```python
from build123d import *

# Parameters (mm, degrees)
SKETCH_1_W          = 5
SKETCH_1_H          = 300
EXTRUDE_1_DEPTH     = 60
SKETCH_2_R          = 5
CUT_EXTRUDE_1_DEPTH = 20


with BuildPart() as part:
    # 草图1 → 凸台-拉伸1 (new body)
    with BuildSketch(Plane.XY):
        Rectangle(SKETCH_1_W, SKETCH_1_H)
    extrude(amount=EXTRUDE_1_DEPTH)

    # 草图2 → 切除-拉伸1 (cut)
    with BuildSketch(Plane(origin=(2.5, 0, 0), x_dir=(0, 0, -1), z_dir=(1, 0, 0))):
        with Locations((-30, -100)):
            Circle(SKETCH_2_R)
    extrude(amount=-CUT_EXTRUDE_1_DEPTH, mode=Mode.SUBTRACT)


solid = part.part
```
Design review of the part built by this model. Coordinates are the model's own, in mm. Give positions to 0.01 mm unless a question says otherwise; leave off trailing zeros. Order: outer loops, then holes, each group sorted by start corner. A loop starts at its lowest first (then second) coordinate and runs counter-clockwise, first axis right, second up. Notation, with made-up numbers: M 83,7 L 98,7 A22 ccw 98,25 Z; hole C 24.5,-34.5 d3. An arc over 180 degrees is marked long. One line per question, with ' | ' between items. Start each with the question number.
Q1. For L1, parallel to Y at x = 0.6, z = 30; L2, parallel to Y at x = -0.05, z = 26; L3, parallel to Z at x = -0.6, y = -102, list the stretches that pass through material, from the lowest coordinate up. Write a range as [from, to].
Q2. We need section A-A (z = 30). Write out the cut boundary in (x, y).
Q3. The part is to be moulded in two halves that separate along Z. For faces 1 (the face through (0.04, -104.88, 31.08)), 2 (the face through (0, 2, 60)), 3 (the face through (0, -150, 30)), say which applies: +Z half, -Z half, draft (parallel to the pull), parting line (faces both ways), or undercut.
Q4. We need section B-B (y = -100). Write out the cut boundary in (x, z), plus the area to 3 significant figures.
Returned:
1) L1: [-150, -105], [-95, 150] | L2: [-150, -103], [-97, 150] | L3: [0, 25.42], [34.58, 60]
2) outline: M -2.5,-150 L 2.5,-150 L 2.5,-105 L -2.5,-105 Z; M -2.5,-95 L 2.5,-95 L 2.5,150 L -2.5,150 Z
3) face 1: undercut | face 2: +Z half | face 3: draft
4) outline: M -2.5,0 L 2.5,0 L 2.5,25 L -2.5,25 Z; M -2.5,35 L 2.5,35 L 2.5,60 L -2.5,60 Z | area: 250 mm2
